Geometry check sheet. Reference: the model listing, model coordinates, mm. Face numbers are marked on the shaded views. A direction names the side the tool comes from. Round coordinates to 2 decimals unless told otherwise and drop trailing zeros. Write each loop counter-clockwise with the first axis right and the second up, starting at its lowest first coordinate (ties: lowest second). Pieces come first, ordered by that corner, then holes.
Item 1: Cross-section at A-A (y = 0). Enter the section's corners in (x, z), then the cut area to 3 significant figures.
Item 2: Depth check by flat-ended pin: P1, Ø8, axis at x = 43, z = 11, coming from the -Y side; P2, Ø4, axis at x = 92.5, y = -6, coming from the +Z side; P3, Ø20.5, axis at y = 15, z = 10, coming from the +X side. Enter the tip coordinate at first touch or a pass-through.
Item 3: Cross-section at D-D (x = 52). Enter the section's corners in (y, z).
Item 4: Cross-section at C-C (x = 13). Enter the section's corners in (y, z), then the cut area to 3 significant figures.
Item 5: Scan lines: probe 1 along X at (y, z) = (14, 18.5); probe 2 along Z at (x, y) = (62, -0.5); probe 3 along X at (y, z) = (1.5, 15). Record each from-to range of solid material in increasing order.
Item 6: Access from +Z, -Z, +X, -X, +Y, -Y to the whole of each face (thin tool, end or side, straight path). Record for the marked faces 1 and 2.
from build123d import *

# Parameters (mm, degrees)
CHAMFER1_SIZE = 0.5
CHAMFER2_SIZE = 0.5
CHAMFER3_SIZE = 15


with BuildPart() as part:
    # Sketch1 → Revolve1 (revolve)
    with BuildSketch(Plane.XY, mode=Mode.PRIVATE) as revolve1_sk:
        Polygon((0, 0), (0, 35), (6, 35), (6, 8), (54, 8), (54, 5), (124, 5), (124, 0), align=None)
    revolve(revolve1_sk.sketch.rotate(Axis((0, 0, 0), (1, 0, 0)), 90), axis=Axis((0, 0, 0), (1, 0, 0)))

    # Chamfer1
    chamfer1_edges = [part.edges().sort_by_distance(p)[0] for p in [
        (54, 0, -8),
        (6, 0, -35),
        (0, 0, -35),
    ]]
    chamfer(chamfer1_edges, length=CHAMFER1_SIZE)

    # Chamfer2
    chamfer2_edges = [part.edges().sort_by_distance(p)[0] for p in [
        (124, 0, -5),
    ]]
    chamfer(chamfer2_edges, length=CHAMFER2_SIZE)

    # Chamfer3
    chamfer3_edges = [part.edges().sort_by_distance(p)[0] for p in [
        (6, 0, -8),
    ]]
    chamfer(chamfer3_edges, length=CHAMFER3_SIZE)


solid = part.part
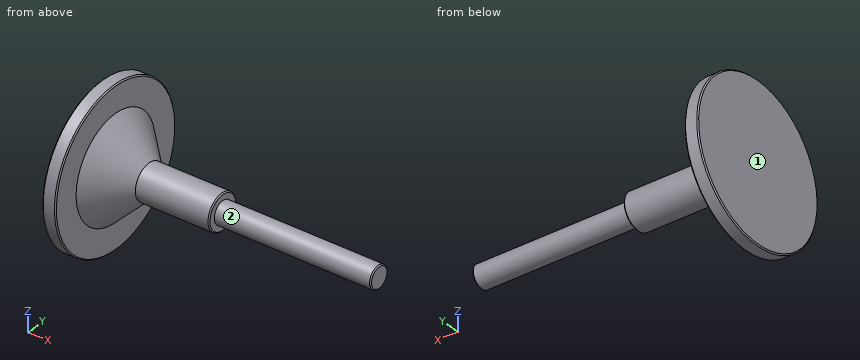
Resolved:
1. outline: (0, -34.5) - (0.5, -35) - (5.5, -35) - (6, -34.5) - (6, -23) - (21, -8) - (53.5, -8) - (54, -7.5) - (54, -5) - (123.5, -5) - (124, -4.5) - (124, 4.5) - (123.5, 5) - (54, 5) - (54, 7.5) - (53.5, 8) - (21, 8) - (6, 23) - (6, 34.5) - (5.5, 35) - (0.5, 35) - (0, 34.5) - close
1. area: 2,110 mm2
2. P1: stops at y = -3.87
2. P2: stops at z = 3
2. P3: stops at x = 53.72
3. outline: circle Ø16 at (0, 0)
4. outline: circle Ø32 at (0, 0)
4. area: 804 mm2
5. probe 1: x = 0 to 6
5. probe 2: z = -4.97 to 4.97
5. probe 3: x = 0 to 13.93
6. face 1: +Z, -Z, -X, +Y, -Y
6. face 2: +X
